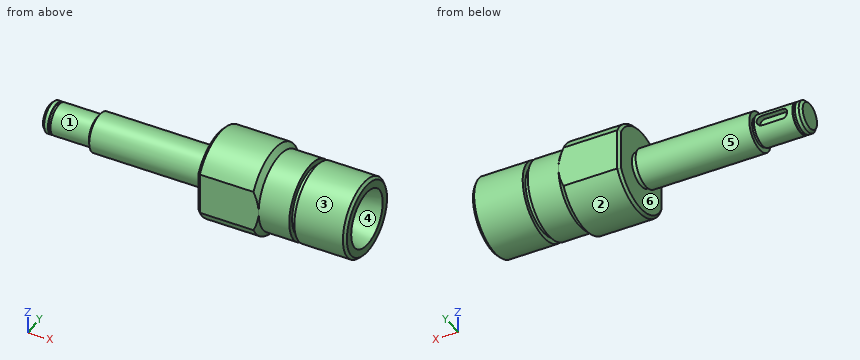
```python
from build123d import *

# Parameters (mm, degrees)
CUT_EXTRUDE1_START = 3.5
CUT_EXTRUDE1_DEPTH = 10
CUT_EXTRUDE2_REACH = 72.242
CHAMFER1_SIZE      = 1
CHAMFER2_SIZE      = 1


with BuildPart() as part:
    # Sketch1 → Revolve1 (revolve)
    with BuildSketch(Plane.XY):
        Polygon((0, 0), (0, 6), (2.5, 6), (2.5, 5.5), (3.5, 5.5), (3.5, 6), (18.5, 6), (18.5, 5.5), (19.5, 5.5), (19.5, 7.5), (64, 7.5), (64, 6.5), (66, 6.5), (66, 17), (88, 17), (90, 15), (102, 15), (102, 13), (104, 13), (104, 15), (124, 15), (124, 0), align=None)
    revolve(axis=Axis((124, 0, 0), (-1, 0, 0)))

    # Sketch3 → Cut-Extrude1 (cut)
    with BuildSketch(Plane(origin=(0, 0, 0), x_dir=(1, 0, 0), z_dir=(0, 1, 0)).offset(CUT_EXTRUDE1_START)):
        with BuildLine():
            Line((15.5, -2), (7.5, -2))
            ThreePointArc((7.5, -2), (5.5, 0), (7.5, 2))
            Line((7.5, 2), (15.5, 2))
            ThreePointArc((15.5, 2), (17.5, 0), (15.5, -2))
        make_face()
    extrude(amount=CUT_EXTRUDE1_DEPTH, mode=Mode.SUBTRACT)

    # Cut-Extrude2: up to this cone (the profile starts inside it)
    cut_extrude2_end = Plane(origin=(66, 0, 0), z_dir=(-1, 0, 0)).offset(-38.999999) * Cone(1e-06, 150.742, 150.741999, align=(Align.CENTER, Align.CENTER, Align.MIN), mode=Mode.PRIVATE)
    # Sketch6 → Cut-Extrude2 (cut, up to the surface)
    with BuildSketch(Plane.ZY.offset(-66), mode=Mode.PRIVATE) as cut_extrude2_sk1:
        with BuildLine():
            Line((-8, 15), (8, 15))
            ThreePointArc((8, 15), (0, 17), (-8, 15))
        make_face()
    cut_extrude2_tool1 = extrude(cut_extrude2_sk1.sketch, amount=-CUT_EXTRUDE2_REACH, mode=Mode.PRIVATE) & cut_extrude2_end
    add(cut_extrude2_tool1.solids().sort_by_distance((66, 15.804176, 0))[0], mode=Mode.SUBTRACT)
    # Sketch6 → Cut-Extrude2 (cut, up to the surface)
    with BuildSketch(Plane.ZY.offset(-66), mode=Mode.PRIVATE) as cut_extrude2_sk2:
        with BuildLine():
            Line((-8, -15), (8, -15))
            ThreePointArc((8, -15), (0, -17), (-8, -15))
        make_face()
    cut_extrude2_tool2 = extrude(cut_extrude2_sk2.sketch, amount=-CUT_EXTRUDE2_REACH, mode=Mode.PRIVATE) & cut_extrude2_end
    add(cut_extrude2_tool2.solids().sort_by_distance((66, -15.804176, 0))[0], mode=Mode.SUBTRACT)

    # Chamfer1
    chamfer1_edges = [part.edges().sort_by_distance(p)[0] for p in [
        (124, -15, 0),
        (66, 0, 17),
        (0, -6, 0),
        (66, 0, -17),
        (66, 15, 0),
        (66, -15, 0),
    ]]
    chamfer(chamfer1_edges, length=CHAMFER1_SIZE)

    # Sketch7 → Cut-Revolve1 (revolve, cut)
    with BuildSketch(Plane.XY, mode=Mode.PRIVATE) as cut_revolve1_sk:
        Polygon((124, 11), (108, 6.712812921), (108, 9.5), (103, 9.5), (103, 9), (97, 9), (97, 9.5), (92, 9.5), (92, 7), (76, 7), (71.958548116, 0), (124, 0), align=None)
    revolve(cut_revolve1_sk.sketch.rotate(Axis((71.958548116, 0, 0), (1, 0, 0)), 180), axis=Axis((71.958548116, 0, 0), (1, 0, 0)), mode=Mode.SUBTRACT)

    # Chamfer2
    chamfer2_edges = [part.edges().sort_by_distance(p)[0] for p in [
        (92, 7, 0),
    ]]
    chamfer(chamfer2_edges, length=CHAMFER2_SIZE)


solid = part.part
```
Geometry: final body of the model. Coordinates: model frame, mm. Face numbers are marked on the shaded views. A direction names the side the tool comes from. Coordinates: 2 decimals unless noted, no trailing zeros. Loops run counter-clockwise (first coordinate to the right, second up) from the corner with the lowest first, then second, coordinate; pieces in that order, holes last. Notation, with made-up numbers: (87.25, -9.5) -> (97.25, -9.5) arc R11 ccw to (97.25, -3.5) -> close; hole circle Ø9 at (80.25, 46). An arc over 180 degrees is marked (long way). Use a Markdown table: item, result. Add a question column.
(1) Access query for the marked faces 1, 2 and 3. Directions: +Z, -Z, +X, -X, +Y, -Y. A direction counts if a zero-diameter tool reaches every point of the face in a straight line with its end or side. Return the directions, or none.
(2) Section query A-A, the plane x = 26. Return loops of the section in (y, z), plus the area to 3 significant figures.
(3) Pin query (flat end, axial travel): pin 1 Ø3.5 at (y, z) = (2.5, 1.5) entering from -X; pin 2 Ø1.2 at (x, z) = (8.5, 1) entering from +Y; pin 3 Ø3 at (x, y) = (82, -10) entering from -Z; pin 4 Ø0.6 at (x, y) = (11.5, 5) entering from +Z. Return the tip coordinate at first contact, or that it passes through.
(4) Section query C-C, the plane x = 12.5. Return loops of the section in (y, z).
(5) Mould query, pull axis Y, two halves, no side actions, for the marked faces 4, 5 and 6. Classes: pulls with the +Y half, pulls with the -Y half, needs draft (parallel to the pull), parting line crosses it, or undercut.
(6) Section query B-B, the plane x = 114.5. Return loops of the section in (y, z).
(7) Line query: line 1 along Z through (x, y) = (105.9, 0); line 2 along Z through (x, y) = (98.9, 0); line 3 along X through (y, z) = (4, 10.5). Output: solid intervals per line, ascending.
Answer:
| question | item | result |
|---|---|---|
| 1 | face 1 | -X |
| 1 | face 2 | -Z, +X, -X |
| 1 | face 3 | +X |
| 2 | outline | circle Ø15 at (0, 0) |
| 2 | area | 177 mm^2 |
| 3 | pin 1 | stops at x = 0 |
| 3 | pin 2 | stops at y = 3.5 |
| 3 | pin 3 | stops at z = -14.72 |
| 3 | pin 4 | stops at z = 3.73 |
| 4 | outline | (3.5, -2) -> (3.5, 2) -> (5.66, 2) arc R6 ccw (long way) to (5.66, -2) -> close |
| 5 | face 4 | undercut |
| 5 | face 5 | parting line crosses it |
| 5 | face 6 | needs draft |
| 6 | outline | circle Ø30 at (0, 0); hole circle Ø16.91 at (0, 0) |
| 7 | line 1 | z = -15 to -9.5, 9.5 to 15 |
| 7 | line 2 | z = -15 to -9, 9 to 15 |
| 7 | line 3 | x = 66 to 124 |
